Design review of the part built by this model. Coordinates are the model's own, in mm. A direction names the side the tool comes from. Give positions to 0.01 mm unless a question says otherwise; leave off trailing zeros. Order: outer loops, then holes, each group sorted by start corner. A loop starts at its lowest first (then second) coordinate and runs counter-clockwise, first axis right, second up. Notation, with made-up numbers: (54.25, 19.25) -> (66.25, 19.25) arc R32 cw to (66.25, 45.25) -> close; hole circle Ø4 at (-29, -16.5). An arc over 180 degrees is marked (long way). One line per item, written item: value. Start each with the question number.
1) Wall thickness on line 1 along Y through (x, z) = (0, 5.5); line 2 along Y through (x, z) = (3, 9); line 3 along X through (y, z) = (21.25, 0): over which ranges is each line inside the solid? List them lowest first. Write a range as from..to.
2) Consider section C-C (x = 0). State how many separate pieces and enclosed holes the cut face has, plus the area to 4 significant figures.
3) The part is to be moulded in two halves that separate along Z. For faces 1 (the face through (-1.5, 22.4, -4.77)), 2 (the face through (-8.2, 21.5, 0)), 3 (the face through (3.06, 23.53, -7.39)), 4 (the face through (-0.751, 7.395, -2.385)), say which applies: released by +Z, released by -Z, zero draft, split by the parting line, or undercut.
4) Consider section A-A (y = 3). State the section outline as (x, z) points.
5) For pin 1 (5 mm diameter, centred on x = -0.5, z = 0, fed in from +Y); pin 2 (4 mm diameter, centred on x = 6.5, y = 11, fed in from +Z); pin 3 (2 mm diameter, centred on y = 9.5, z = -3.5, fed in from +X); pin 4 (4.5 mm diameter, centred on x = 0, z = 0, fed in from -Y), all flat-tipped, find the tip position at first contact; note any pin that passes through.
6) Tool access review of faces 5 (the face through (-8.2, 8.5, 0)), 6 (the face through (0, 28, 10)), 7 (the face through (1.5, 23.43, 6.36)): name each direction out of +Z, -Z, +X, -X, +Y, -Y from which nothing blocks a thin tool from reaching the whole face with its end or side.
from build123d import *

# Parameters (mm, degrees)
CUT_EXTRUDE1_REACH      = 35.166
CUT_EXTRUDE1_END_RADIUS = 8
SKETCH2_R               = 1.5


with BuildPart() as part:
    # Sketch1 → Revolve1 (revolve)
    with BuildSketch(Plane.XY, mode=Mode.PRIVATE) as revolve1_sk:
        Polygon((2.5, 15), (2.5, 0), (10, 0), (10, 4.5), (8, 4.5), (8, 8.5), (10, 8.5), (10, 13), (8, 13), (8, 17), (10, 17), (10, 21.5), (8, 21.5), (8, 25.5), (10, 25.5), (10, 30), (5, 30), (5, 15), align=None)
    revolve(revolve1_sk.sketch.rotate(Axis((0, 0, 0), (0, 1, 0)), 90), axis=Axis((0, 0, 0), (0, 1, 0)))

    # Cut-Extrude1: up to this cylinder (the profile starts inside it)
    cut_extrude1_end = Plane(origin=(0, 15, 0), z_dir=(0, -1, 0)) * Cylinder(CUT_EXTRUDE1_END_RADIUS, 104.332, mode=Mode.PRIVATE)
    # Sketch2 → Cut-Extrude1 (cut, up to the surface)
    with BuildSketch(Plane.XY, mode=Mode.PRIVATE) as cut_extrude1_sk1:
        with Locations(Location((0, 23.5, 0), (0, 0, 180))):
            Circle(SKETCH2_R)
    cut_extrude1_tool1 = extrude(cut_extrude1_sk1.sketch, amount=CUT_EXTRUDE1_REACH, mode=Mode.PRIVATE) & cut_extrude1_end
    add(cut_extrude1_tool1.solids().sort_by_distance((0, 23.5, 0))[0], mode=Mode.SUBTRACT)
    # Sketch2 → Cut-Extrude1 (cut, up to the surface)
    with BuildSketch(Plane.XY, mode=Mode.PRIVATE) as cut_extrude1_sk2:
        with Locations(Location((0, 6.5, 0), (0, 0, 180))):
            Circle(SKETCH2_R)
    cut_extrude1_tool2 = extrude(cut_extrude1_sk2.sketch, amount=CUT_EXTRUDE1_REACH, mode=Mode.PRIVATE) & cut_extrude1_end
    add(cut_extrude1_tool2.solids().sort_by_distance((0, 6.5, 0))[0], mode=Mode.SUBTRACT)


solid = part.part
Checked values:
1. line 1: y = 0..5, 8..22, 25..30
1. line 2: y = 0..4.5, 8.5..13, 17..21.5, 25.5..30
1. line 3: x = -10..-5, 5..10
2. separate pieces: 4
2. enclosed holes: 0
2. area: 301.5 mm^2
3. face 1: undercut
3. face 2: zero draft
3. face 3: split by the parting line
3. face 4: undercut
4. outline: circle Ø20 at (0, 0); hole circle Ø5 at (0, 0)
5. pin 1: stops at y = 15
5. pin 2: stops at z = 8.93
5. pin 3: stops at x = 9.68
5. pin 4: passes through
6. face 5: none
6. face 6: +Y, -Y
6. face 7: +Z
